```python
from build123d import *

# Parameters (mm, degrees)
EXTRUDE_1_DEPTH     = 30
MM_1_D              = 3
CUT_EXTRUDE_1_DEPTH = 3.5
CUT_EXTRUDE_2_REACH = 19.682
SKETCH_15_R         = 1.1
CUT_EXTRUDE_3_DEPTH = 5


with BuildPart() as part:
    # 草图2 → 凸台-拉伸1 (new body)
    with BuildSketch(Plane(origin=(15, 0, 0), x_dir=(0, 0, -1), z_dir=(1, 0, 0))):
        with BuildLine():
            Line((0, -3.5), (1, -2.5))
            Line((1, -2.5), (8, -2.5))
            Line((8, -2.5), (8, -5))
            Line((8, -5), (6.535231383, -5))
            ThreePointArc((6.535231383, -5), (5.073455672, -5.471894537), (4.163523138, -6.709430585))
            Line((4.163523138, -6.709430585), (3.710344828, -8.068965517))
            Line((3.710344828, -8.068965517), (0.751935513, -9.794704284))
            ThreePointArc((0.751935513, -9.794704284), (0.250969637, -9.79638591), (0, -9.362814834))
            Line((0, -9.362814834), (0, -3.5))
        make_face()
    extrude(amount=-EXTRUDE_1_DEPTH)

    # 大小mm 暗销孔1 (through all)
    with Locations(Plane(origin=(0, -2.5, 0), x_dir=(1, 0, 0), z_dir=(0, 1, 0))):
        with Locations((6, 5.3), (-6, 5.3)):
            Hole(MM_1_D / 2)

    # 草图13 → 切除-拉伸1 (cut)
    with BuildSketch(Plane(origin=(0, -8.5, 0), x_dir=(1, 0, 0), z_dir=(0, 1, 0))):
        with BuildLine():
            ThreePointArc((10.927039915, 6.535231383), (12.5, 3.3), (14.072960085, 6.535231383))
            ThreePointArc((14.072960085, 6.535231383), (12.5, 7.186772784), (10.927039915, 6.535231383))
        make_face()
    extrude(amount=CUT_EXTRUDE_1_DEPTH, mode=Mode.SUBTRACT)

    # 草图14 → 切除-拉伸2 (cut, up to next)
    with BuildSketch(Plane.XZ.offset(5), mode=Mode.PRIVATE) as cut_extrude_2_sk1:
        with BuildLine():
            ThreePointArc((-10.927039915, -6.535231383), (-12.5, -3.3), (-14.072960085, -6.535231383))
            ThreePointArc((-14.072960085, -6.535231383), (-12.5, -7.186772784), (-10.927039915, -6.535231383))
        make_face()
    cut_extrude_2_tool1 = extrude(cut_extrude_2_sk1.sketch, amount=CUT_EXTRUDE_2_REACH, mode=Mode.PRIVATE) & part.part
    add(cut_extrude_2_tool1.solids().sort_by_distance((-12.5, -5, -5.261226))[0], mode=Mode.SUBTRACT)

    # 草图15 → 切除-拉伸3 (cut)
    with BuildSketch(Plane.XZ.offset(5)):
        with Locations(Location((12.5, -5.3, 0), (0, 0, 270))):
            Circle(SKETCH_15_R)
        with Locations(Location((-12.5, -5.3, 0), (0, 0, 270))):
            Circle(SKETCH_15_R)
    extrude(amount=-CUT_EXTRUDE_3_DEPTH, mode=Mode.SUBTRACT)


solid = part.part
```
Input: part model. Units: mm. Frame: model coordinates. Round coordinates to 2 decimals unless told otherwise and drop trailing zeros. Order: outer loops, then holes, each group sorted by start corner. A loop starts at its lowest first (then second) coordinate and runs counter-clockwise, first axis right, second up. Notation, with made-up numbers: (61, 89.5) - (105, 89.5) arc R22 ccw to (105, 109.5) - close; hole circle Ø8 at (-1.5, 23). An arc over 180 degrees is marked (long way). Answer in a Markdown table with one row per item.
Item 1: Pin query (flat end, axial travel): pin 1 (2.5 mm diameter, centred on x = 12.5, z = -5.3, fed in from -Y); pin 2 (2.5 mm diameter, centred on x = 5.5, z = -6.5, fed in from -Y); pin 3 (3 mm diameter, centred on x = 3.5, z = -6, fed in from -Y); pin 4 (1.8 mm diameter, centred on x = -6, z = -5.3, fed in from +Y). Return the tip coordinate at first contact, or that it passes through.
Model answer:
| item | result |
|---|---|
| pin 1 | stops at y = -5 |
| pin 2 | stops at y = -5.15 |
| pin 3 | stops at y = -6.05 |
| pin 4 | passes through |
Item 2: Section query D-D (z = -3). Return the cut outline in (x, y).
Model answer:
| item | result |
|---|---|
| outline | (-15, -8.48) - (15, -8.48) - (15, -2.5) - (-15, -2.5) - close |
Item 3: Section query A-A (x = -12.5). Return the cut outline in (y, z), then the cut area to 3 significant figures.
Model answer:
| item | result |
|---|---|
| outline | (-9.79, -0.75) - (-8.31, -3.3) - (-5, -3.3) - (-5, -4.2) - (-2.5, -4.2) - (-2.5, -1) - (-3.5, 0) - (-9.36, 0) arc R0.5 ccw to start; (-5, -8) - (-2.5, -8) - (-2.5, -6.4) - (-5, -6.4) - close |
| area | 27.9 mm² |
Item 4: Line query: line 1 (X direction, y = -4.7, z = -5.3); line 2 (Y direction, x = -11.5, z = -6); line 3 (Z direction, x = -12.5, y = -7.1). Output: solid intervals per line, ascending.
Model answer:
| item | result |
|---|---|
| line 1 | x = -15 to -13.6, -11.4 to -7.5, -4.5 to 4.5, 7.5 to 11.4, 13.6 to 15 |
| line 2 | y = -5 to -2.5 |
| line 3 | z = -3.3 to 0 |
Item 5: Section query C-C (x = 6). Return the cut outline in (y, z).
Model answer:
| item | result |
|---|---|
| outline | (-9.79, -0.75) - (-8.07, -3.71) - (-7.8, -3.8) - (-2.5, -3.8) - (-2.5, -1) - (-3.5, 0) - (-9.36, 0) arc R0.5 ccw to start; (-5, -8) - (-2.5, -8) - (-2.5, -6.8) - (-5, -6.8) - close |
Item 6: Section query B-B (z = -5.75). Return the cut outline in (x, y), then the cut area to 3 significant figures.
Model answer:
| item | result |
|---|---|
| outline | (-15, -5.13) - (-14.45, -5.13) - (-14.45, -5) - (-13.5, -5) - (-13.5, -2.5) - (-15, -2.5) - close; (-11.5, -5) - (-10.55, -5) - (-10.55, -5.13) - (-7.43, -5.13) - (-7.43, -2.5) - (-11.5, -2.5) - close; (-4.57, -5.13) - (4.57, -5.13) - (4.57, -2.5) - (-4.57, -2.5) - close; (7.43, -5.13) - (10.55, -5.13) - (10.55, -5) - (11.5, -5) - (11.5, -2.5) - (7.43, -2.5) - close; (13.5, -5) - (14.45, -5) - (14.45, -5.13) - (15, -5.13) - (15, -2.5) - (13.5, -2.5) - close |
| area | 52.7 mm² |
